Geometry: see drawing. Coordinates: mm, zero at the bounding-box minimum. Round coordinates to 2 decimals unless told otherwise and drop trailing zeros. Loops run counter-clockwise (first coordinate to the right, second up) from the corner with the lowest first, then second, coordinate; pieces in that order, holes last. Notation, with made-up numbers: (-19, 74) -> (-9, 74) arc R13 ccw to (-9, 90) -> close; hole circle Ø6 at (6, 12). An arc over 180 degrees is marked (long way). Write item = value, one per line.
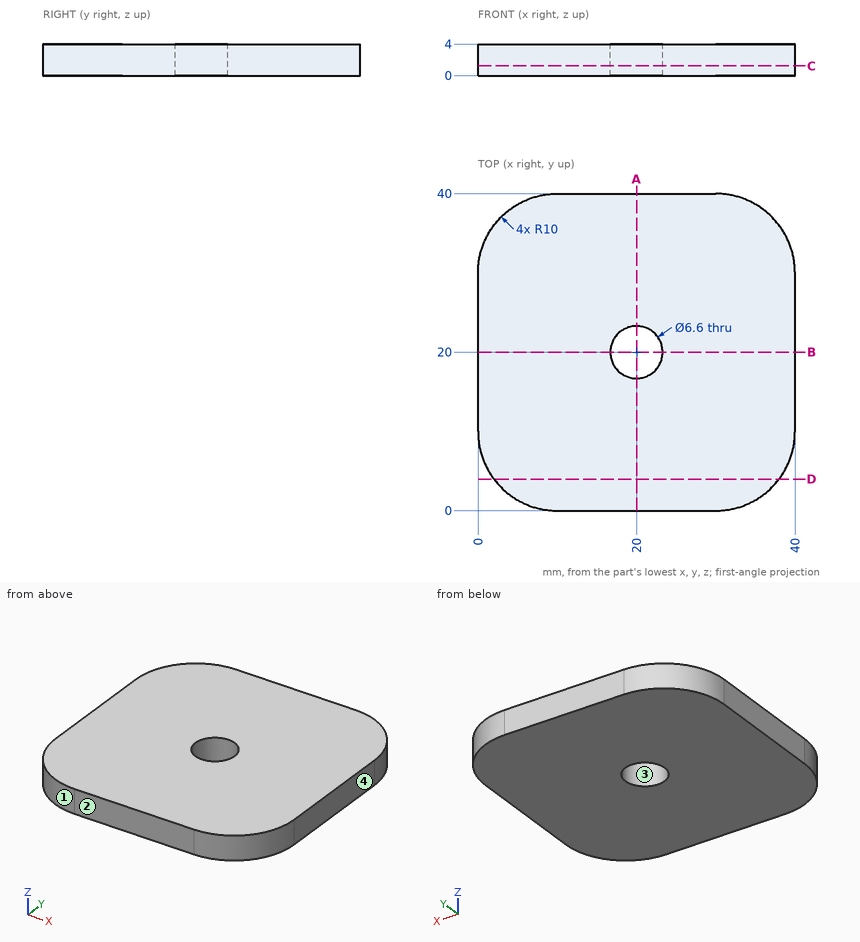
1. Section query D-D (y = 4). Return the cut outline in (x, z).
Evaluation:
outline = (2, 0) -> (38, 0) -> (38, 4) -> (2, 4) -> close
2. Line query: probe 1 along Y at (x, z) = (20, 3.05); probe 2 along X at (y, z) = (23, 1.95); probe 3 along Y at (x, z) = (22.5, 0.5). Output: solid intervals per line, ascending. Write a range as from..to.
Evaluation:
probe_1 = 0..16.7, 23.3..40
probe_2 = 0..18.63, 21.37..40
probe_3 = 0..17.85, 22.15..40
3. Section query C-C (z = 1.25). Return the cut outline in (x, y), then the cut area to 3 significant figures.
Evaluation:
outline = (0, 10) arc R10 ccw to (10, 0) -> (30, 0) arc R10 ccw to (40, 10) -> (40, 30) arc R10 ccw to (30, 40) -> (10, 40) arc R10 ccw to (0, 30) -> close; hole circle Ø6.6 at (20, 20)
area = 1,480 mm²
4. Mould query, pull axis X, two halves, no side actions, for the marked faces 1, 2, 3 and 4. Classes: released by +X, released by -X, zero draft, split by the parting line, or undercut.
Evaluation:
face_1 = released by -X
face_2 = zero draft
face_3 = undercut
face_4 = released by +X
5. Section query A-A (x = 20). Return the cut outline in (y, z).
Evaluation:
outline = (0, 0) -> (16.7, 0) -> (16.7, 4) -> (0, 4) -> close; (23.3, 0) -> (40, 0) -> (40, 4) -> (23.3, 4) -> close
